Verification items for the finished model (mm, model axes). A direction names the side the tool comes from. Give positions to 0.01 mm unless a question says otherwise; leave off trailing zeros. Write each loop counter-clockwise with the first axis right and the second up, starting at its lowest first coordinate (ties: lowest second). Pieces come first, ordered by that corner, then holes. Notation, with made-up numbers: M 85,66.5 L 141,66.5 A21 cw 141,85.5 Z; hole C -6,71.5 d7. An arc over 180 degrees is marked long. Answer as a JSON object with one key per item and string values.
```python
from build123d import *

# Parameters (mm, degrees)
SKETCH1_W           = 105
SKETCH1_H           = 12
BOSS_EXTRUDE1_DEPTH = 8
CHAMFER1_SIZE       = 2
SKETCH2_R           = 2.25
CUT_EXTRUDE1_DEPTH  = 10
CUT_EXTRUDE2_DEPTH  = 10


with BuildPart() as part:
    # Sketch1 → Boss-Extrude1 (new body)
    with BuildSketch(Plane(origin=(0, 0, 0), x_dir=(1, 0, 0), z_dir=(0, 1, 0))):
        with Locations((52.5, 6)):
            Rectangle(SKETCH1_W, SKETCH1_H)
    extrude(amount=BOSS_EXTRUDE1_DEPTH)

    # Chamfer1
    chamfer1_edges = [part.edges().sort_by_distance(p)[0] for p in [
        (0, 4, -12),
        (105, 4, -12),
        (105, 4, 0),
        (0, 4, 0),
    ]]
    chamfer(chamfer1_edges, length=CHAMFER1_SIZE)

    # Sketch2 → Cut-Extrude1 (cut)
    with BuildSketch(Plane(origin=(0, 8, 0), x_dir=(1, 0, 0), z_dir=(0, 1, 0))):
        with Locations(Location((7.5, 6, 0), (0, 0, 270))):
            Circle(SKETCH2_R)
        with Locations(Location((97.5, 6, 0), (0, 0, 90))):
            Circle(SKETCH2_R)
    extrude(amount=-CUT_EXTRUDE1_DEPTH, mode=Mode.SUBTRACT)

    # Sketch3 → Cut-Extrude2 (cut)
    with BuildSketch(Plane(origin=(0, 8, 0), x_dir=(1, 0, 0), z_dir=(0, 1, 0))):
        with BuildLine():
            Line((5.25, 4), (5.25, 8))
            ThreePointArc((5.25, 8), (7.5, 10.25), (9.75, 8))
            Line((9.75, 8), (9.75, 4))
            ThreePointArc((9.75, 4), (7.5, 1.75), (5.25, 4))
        make_face()
        with BuildLine():
            Line((99.75, 4), (99.75, 8))
            ThreePointArc((99.75, 8), (97.5, 10.25), (95.25, 8))
            Line((95.25, 8), (95.25, 4))
            ThreePointArc((95.25, 4), (97.5, 1.75), (99.75, 4))
        make_face()
    extrude(amount=-CUT_EXTRUDE2_DEPTH, mode=Mode.SUBTRACT)


solid = part.part
```
1) Section check A-A on x = 97.5. Record the boundary of the cut face in (y, z).
Completed:
{"outline": "M 0,-12 L 8,-12 L 8,-10.25 L 0,-10.25 Z; M 0,-1.75 L 8,-1.75 L 8,0 L 0,0 Z"}
2) Release check for a two-part mould opening along Z. For faces 3 (the face through (5.25, 4, -6)), 4 (the face through (52, 4, -12)), 5 (the face through (105, 4, -6)) record: pulls with the +Z half, pulls with the -Z half, needs draft (parallel to the pull), parting line crosses it, or undercut.
Completed:
{"face 3": "undercut", "face 4": "pulls with the -Z half", "face 5": "needs draft"}
3) Go/stop test with a flat-tipped pin: pin 1 (2 mm diameter, centred on y = 2.5, z = -1.5, fed in from +X). Record where the tip stops, or that it passes through.
Completed:
{"pin 1": "stops at x = 105"}
4) Thickness scan on L1, parallel to X at y = 2, z = -7.5; L2, parallel to Z at x = 8, y = 4.25. Record the ranges inside material, lowest first.
Completed:
{"L1": "x = 0 to 5.25, 9.75 to 95.25, 99.75 to 105", "L2": "z = -12 to -10.19, -1.81 to 0"}
5) Access from +Z, -Z, +X, -X, +Y, -Y to the whole of each face (thin tool, end or side, straight path). Record for faces 1 (the face through (97.45, 4.06, -1.75)), 2 (the face through (1, 4, -11)).
Completed:
{"face 1": "+Y, -Y", "face 2": "-Z, -X, +Y, -Y"}
6) Section check B-B on y = 2. Record the boundary of the cut face in (x, z).
Completed:
{"outline": "M 0,-10 L 2,-12 L 103,-12 L 105,-10 L 105,-2 L 103,0 L 2,0 L 0,-2 Z; hole M 5.25,-8 A2.25 ccw 9.75,-8 L 9.75,-4 A2.25 ccw 5.25,-4 Z; hole M 95.25,-8 A2.25 ccw 99.75,-8 L 99.75,-4 A2.25 ccw 95.25,-4 Z"}
